Could you check a few things on this model? Use its own coordinates, in mm. Give positions to 0.01 mm unless a question says otherwise; leave off trailing zeros. Loops run counter-clockwise (first coordinate to the right, second up) from the corner with the lowest first, then second, coordinate; pieces in that order, holes last.
1. For P1, Ø8, axis at x = 5.5, z = -12.5, coming from the -Y side; P2, Ø4, axis at x = 17.5, z = 40, coming from the +Y side, each with a flat end and sliding along its axis, tell me the tip position at first contact or that it passes through.
2. Imagine slicing it at A-A (z = 0). List the corners of the cut face in (x, y) for me, plus the area to 3 significant figures.
3. Imagine slicing it at B-B (x = 80). List the corners of the cut face in (y, z) for me.
4. I need wall thicknesses on line 1 along Z through (x, y) = (-17.5, 2.9); line 2 along X through (y, z) = (1.4, -40); line 3 along X through (y, z) = (1.05, 0). Which ranges of each line are inside material? Lowest first, please.
```python
from build123d import *

# Parameters (mm, degrees)
SKETCH1_W                      = 320
SKETCH1_H                      = 350
BOSS_EXTRUDE1_DEPTH            = 4
F_5_2_5_2_DIAMETER_HOLE1_D     = 5.2
F_5_2_5_2_DIAMETER_HOLE1_DEPTH = 10.1
F_5_2_5_2_DIAMETER_HOLE1_TIP   = 1.562237609
FILLET1_R                      = 10
SKETCH4_R                      = 10
CUT_EXTRUDE1_DEPTH             = 238.151850088


with BuildPart() as part:
    # Sketch1 → Boss-Extrude1 (new body)
    with BuildSketch(Plane(origin=(0, 0, 0), x_dir=(1, 0, 0), z_dir=(0, 1, 0))):
        Rectangle(SKETCH1_W, SKETCH1_H)
    extrude(amount=BOSS_EXTRUDE1_DEPTH)

    # Ø5.2 (5.2) Diameter Hole1
    with Locations(Plane(origin=(0, 4, 0), x_dir=(1, 0, 0), z_dir=(0, 1, 0))):
        with Locations((-17.5, 40), (17.5, -40), (-17.5, -40), (17.5, 40)):
            Hole(F_5_2_5_2_DIAMETER_HOLE1_D / 2, depth=F_5_2_5_2_DIAMETER_HOLE1_DEPTH)
            with Locations((0, 0, -(F_5_2_5_2_DIAMETER_HOLE1_DEPTH + F_5_2_5_2_DIAMETER_HOLE1_TIP / 2))):  # 118° drill point
                Cone(0, F_5_2_5_2_DIAMETER_HOLE1_D / 2, F_5_2_5_2_DIAMETER_HOLE1_TIP, mode=Mode.SUBTRACT)

    # Fillet1
    fillet1_edges = [part.edges().sort_by_distance(p)[0] for p in [
        (-160, 2, -175),
        (160, 2, -175),
        (160, 2, 175),
        (-160, 2, 175),
    ]]
    fillet(fillet1_edges, radius=FILLET1_R)

    # Sketch4 → Cut-Extrude1 (cut, through all)
    with BuildSketch(Plane(origin=(0, 4, 0), x_dir=(1, 0, 0), z_dir=(0, 1, 0))):
        with Locations(Location((80, 0, 0), (0, 0, 270))):
            Circle(SKETCH4_R)
    extrude(amount=-CUT_EXTRUDE1_DEPTH, mode=Mode.SUBTRACT)


solid = part.part
```
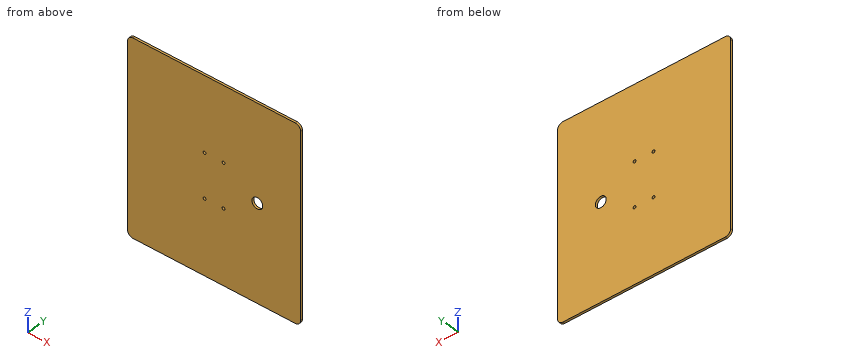
Derived:
1. P1: stops at y = 0
1. P2: passes through
2. outline: (-160, 0) - (70, 0) - (70, 4) - (-160, 4) - close; (90, 0) - (160, 0) - (160, 4) - (90, 4) - close
2. area: 1,200 mm2
3. outline: (0, -175) - (4, -175) - (4, -10) - (0, -10) - close; (0, 10) - (4, 10) - (4, 175) - (0, 175) - close
4. line 1: z = -175 to -42.6, -37.4 to 37.4, 42.6 to 175
4. line 2: x = -160 to -20.1, -14.9 to 14.9, 20.1 to 160
4. line 3: x = -160 to 70, 90 to 160
